For this review, take the finished solid that the model builds, in its own axes (mm). Face numbers are marked on the shaded views. A direction names the side the tool comes from. Coordinates: 2 decimals unless noted, no trailing zeros. Write each loop counter-clockwise with the first axis right and the second up, starting at its lowest first coordinate (ties: lowest second). Pieces come first, ordered by that corner, then holes.
```python
from build123d import *

# Parameters (mm, degrees)
BASE_PLATE_DEPTH              = 10
LOWER_RAIL_DEPTH              = 270
UPPER_BLOCK_DEPTH             = 120
BLOCK_HOLES_AND_SLOT_SKETCH_R = 15
BLOCK_HOLES_AND_SLOT_DEPTH    = 212
BASE_SLOT_COUNTERBORE_DEPTH   = 10
BASE_THROUGH_SLOT_DEPTH       = 68


with BuildPart() as part:
    # Base Plate Sketch → Base Plate (new body)
    with BuildSketch(Plane(origin=(0, 0, 0), x_dir=(1, 0, 0), z_dir=(0, 1, 0))):
        Polygon((145, 0), (145, 60), (-145, 60), (-145, -60), (145, -60), align=None)
    extrude(amount=BASE_PLATE_DEPTH)

    # Lower Rail Sketch → Lower Rail (add)
    with BuildSketch(Plane.ZY.offset(145)):
        Polygon((60, 0), (46.010770255, -30), (-46.010770255, -30), (-60, 0), align=None)
    extrude(amount=-LOWER_RAIL_DEPTH)

    # Upper Block Sketch → Upper Block (add)
    with BuildSketch(Plane(origin=(25, 0, 0), x_dir=(0, 0, -1), z_dir=(1, 0, 0))):
        Polygon((0, 110), (40, 110), (60, 45), (60, 10), (-60, 10), (-60, 45), (-40, 110), align=None)
    extrude(amount=UPPER_BLOCK_DEPTH)

    # Block Holes and Slot Sketch → Block Holes and Slot (cut)
    with BuildSketch(Plane.ZY.offset(-25)):
        with Locations((22.5, 35)):
            Circle(BLOCK_HOLES_AND_SLOT_SKETCH_R)
        with Locations((-22.5, 35)):
            Circle(BLOCK_HOLES_AND_SLOT_SKETCH_R)
        with BuildLine():
            Line((-26, 95), (26, 95))
            ThreePointArc((26, 95), (41, 80), (26, 65))
            Line((26, 65), (-26, 65))
            ThreePointArc((-26, 65), (-41, 80), (-26, 95))
        make_face()
    extrude(amount=-BLOCK_HOLES_AND_SLOT_DEPTH, mode=Mode.SUBTRACT)

    # Base Slot Counterbore Sketch → Base Slot Counterbore (cut)
    with BuildSketch(Plane(origin=(0, 10, 0), x_dir=(1, 0, 0), z_dir=(0, 1, 0))):
        with BuildLine():
            Line((-80, 35), (-25, 35))
            ThreePointArc((-25, 35), (10, 0), (-25, -35))
            Line((-25, -35), (-80, -35))
            ThreePointArc((-80, -35), (-115, 0), (-80, 35))
        make_face()
    extrude(amount=-BASE_SLOT_COUNTERBORE_DEPTH, mode=Mode.SUBTRACT)

    # Base Through Slot Sketch → Base Through Slot (cut)
    with BuildSketch(Plane(origin=(0, 0, 0), x_dir=(1, 0, 0), z_dir=(0, 1, 0))):
        with BuildLine():
            Line((-80, 16), (-25, 16))
            ThreePointArc((-25, 16), (-9, 0), (-25, -16))
            Line((-25, -16), (-80, -16))
            ThreePointArc((-80, -16), (-96, 0), (-80, 16))
        make_face()
    extrude(amount=-BASE_THROUGH_SLOT_DEPTH, mode=Mode.SUBTRACT)


solid = part.part
```
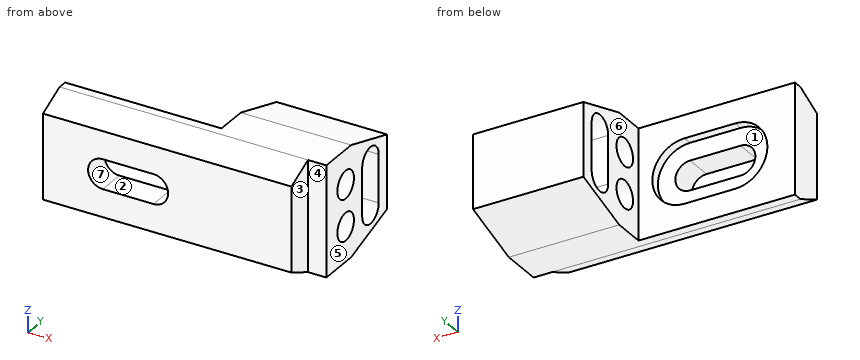
Q1. Add section C-C (x = 58). State the section outline as (y, z) points.
Ans:
outline: (-30, -46.01) - (0, -60) - (45, -60) - (110, -40) - (110, 40) - (45, 60) - (0, 60) - (-30, 46.01) - close; hole circle Ø30 at (35, -22.5); hole circle Ø30 at (35, 22.5); hole (65, -26) arc R15 ccw to (95, -26) - (95, 26) arc R15 ccw to (65, 26) - close
Q2. Add section A-A (x = -50). State the section outline as (y, z) points.
Ans:
outline: (-30, -46.01) - (0, -60) - (10, -60) - (10, -35) - (0, -35) - (0, -16) - (-30, -16) - close; (-30, 16) - (0, 16) - (0, 35) - (10, 35) - (10, 60) - (0, 60) - (-30, 46.01) - close
Q3. Add section B-B (z = 0). State the section outline as (x, y) points.
Ans:
outline: (-145, -30) - (-96, -30) - (-96, 0) - (-115, 0) - (-115, 10) - (-145, 10) - close; (-9, -30) - (125, -30) - (125, 0) - (145, 0) - (145, 65) - (25, 65) - (25, 10) - (10, 10) - (10, 0) - (-9, 0) - close; (25, 95) - (145, 95) - (145, 110) - (25, 110) - close
Q4. Tool access review of the marked faces 1, 2 and 3: name each direction out of +Z, -Z, +X, -X, +Y, -Y from which nothing blocks a thin tool from reaching the whole face with its end or side.
Ans:
face 1: +Y
face 2: +Y, -Y
face 3: +Z, -Z, +X, -Y
Q5. Clearance check with flat-ended pins moving along their axes: pin 1 Ø1.5 at (x, y) = (78, 61) entering from -Z; pin 2 Ø24 at (x, y) = (-63.5, -20.5) entering from -Z; pin 3 Ø9 at (y, z) = (-14.5, 1) entering from +X. State where each tip first meets the part, or that it passes through.
Ans:
pin 1: stops at z = -55.31
pin 2: stops at z = -56.04
pin 3: stops at x = 125
Q6. Add section D-D (y = 28). State the section outline as (x, z) points.
Ans:
outline: (25, -60) - (145, -60) - (145, -35.77) - (25, -35.77) - close; (25, -9.23) - (145, -9.23) - (145, 9.23) - (25, 9.23) - close; (25, 35.77) - (145, 35.77) - (145, 60) - (25, 60) - close
Q7. For probe 1 along Y at (x, z) = (64, -22); probe 2 along Z at (x, y) = (55, 25.5); probe 3 along Y at (x, z) = (-12, 19), list the stretches that pass through material, from the lowest coordinate up.
Ans:
probe 1: y = -30 to 20.01, 49.99 to 65, 95 to 110
probe 2: z = -60 to -34.11, -10.89 to 10.89, 34.11 to 60
probe 3: y = -30 to 0
Q8. Draft analysis for pull direction X (two halves, no side actions). For the marked faces 4, 5, 6 and 7, state which applies: +X half, -X half, draft (parallel to the pull), parting line (faces both ways), or undercut.
Ans:
face 4: draft
face 5: +X half
face 6: -X half
face 7: undercut
